Read the model definition and answer for the solid it produces. Units are mm, in the model's axes. Face numbers are marked on the shaded views. A direction names the side the tool comes from. Give positions to 0.01 mm unless a question says otherwise; leave off trailing zeros. Write each loop counter-clockwise with the first axis right and the second up, starting at its lowest first coordinate (ties: lowest second). Pieces come first, ordered by that corner, then holes. Notation, with made-up numbers: M 13,-20.75 L 44,-20.75 A17 cw 44,8.25 Z; hole C 44.5,-23.5 d11. An arc over 180 degrees is marked long. Answer as CSV lines item,"result". Start each with the question number.
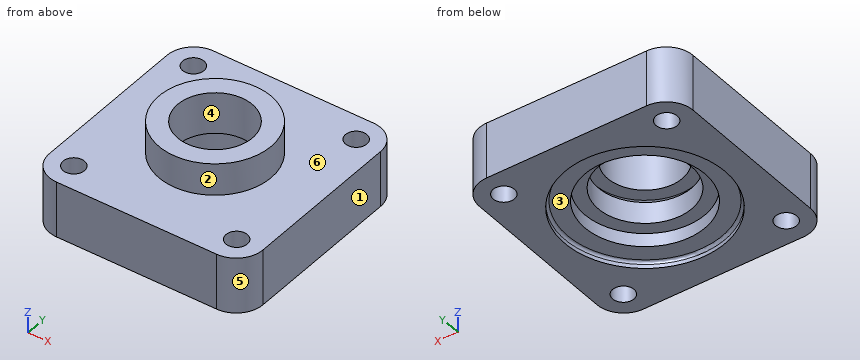
```python
from build123d import *

# Parameters (mm, degrees)
SKETCH_1_W               = 80
SKETCH_1_H               = 80
EXTRUDE_1_DEPTH          = 21
SKETCH_2_R               = 21
EXTRUDE_2_DEPTH          = 12
FILLET_1_R               = 10
SKETCH_6_R               = 4
CUT_EXTRUDE_1_DEPTH      = 21
MIRROR_2_COPY_1_SKETCH_R = 4
MIRROR_2_COPY_1_DEPTH    = 21
FILLET_2_R               = 1
FILLET_3_R               = 1


with BuildPart() as part:
    # 草图1 → 凸台-拉伸1 (new body)
    with BuildSketch(Plane.XY):
        Rectangle(SKETCH_1_W, SKETCH_1_H)
    extrude(amount=EXTRUDE_1_DEPTH)

    # 草图2 → 凸台-拉伸2 (add)
    with BuildSketch(Plane.XY.offset(21)):
        Circle(SKETCH_2_R)
    extrude(amount=EXTRUDE_2_DEPTH)

    # 草图3 → 切除-旋转1 (revolve, cut)
    with BuildSketch(Plane(origin=(0, 0, 0), x_dir=(1, 0, 0), z_dir=(0, 1, 0)), mode=Mode.PRIVATE) as cut_revolve_1_sk:
        Polygon((30, 0), (30, -2.5), (22.5, -2.5), (22.5, -7.5), (17.5, -7.5), (17.5, -15.5), (20, -15.5), (20, -17.5), (14, -17.5), (14, -33), (0, -33), (0, 0), align=None)
    revolve(cut_revolve_1_sk.sketch.rotate(Axis((0, 0, 0), (0, 0, 1)), 180), axis=Axis((0, 0, 0), (0, 0, 1)), mode=Mode.SUBTRACT)

    # 圆角1
    fillet_1_edges = [part.edges().sort_by_distance(p)[0] for p in [
        (40, -40, 10.5),
        (-40, -40, 10.5),
        (-40, 40, 10.5),
        (40, 40, 10.5),
    ]]
    fillet(fillet_1_edges, radius=FILLET_1_R)

    # 草图6 → 切除-拉伸1 (cut)
    with BuildSketch(Plane.XY.offset(21)):
        with Locations((-30.5, 30.5)):
            Circle(SKETCH_6_R)
    cut_extrude_1 = extrude(amount=-CUT_EXTRUDE_1_DEPTH, mode=Mode.SUBTRACT)

    # 镜向1: 切除-拉伸1 across plane
    add(cut_extrude_1.mirror(Plane.ZX), mode=Mode.SUBTRACT)

    # 镜向2: 切除-拉伸1 across plane
    add(cut_extrude_1.mirror(Plane(origin=(0, 0, 0), x_dir=(0, 0, 1), z_dir=(1, 0, 0))), mode=Mode.SUBTRACT)

    # 镜向2 copy 1 sketch → 镜向2 copy 1 (cut)
    with BuildSketch(Plane(origin=(0, 0, 21), x_dir=(-1, 0, 0), z_dir=(0, 0, 1))):
        with Locations((-30.5, 30.5)):
            Circle(MIRROR_2_COPY_1_SKETCH_R)
    extrude(amount=-MIRROR_2_COPY_1_DEPTH, mode=Mode.SUBTRACT)

    # 圆角2
    fillet_2_edges = [part.edges().sort_by_distance(p)[0] for p in [
        (30, 0, 2.5),
    ]]
    fillet(fillet_2_edges, radius=FILLET_2_R)

    # 圆角3
    fillet_3_edges = [part.edges().sort_by_distance(p)[0] for p in [
        (20, 0, 17.5),
    ]]
    fillet(fillet_3_edges, radius=FILLET_3_R)


solid = part.part
```
1. Find the intervals of material crossed by line 1 (Y direction, x = -30.5, z = 12.25); line 2 (X direction, y = 30, z = 12); line 3 (X direction, y = -32, z = 18.5), in increasing order. Write a range as [from, to].
2. Determine the mould class of the marked faces 4, 5 and 6 for opening direction Y: +Y half, -Y half, draft (parallel to the pull), parting line (faces both ways), or undercut.
3. Given pin 1 (19 mm diameter, centred on x = 3.5, y = -9, fed in from -Z); pin 2 (4 mm diameter, centred on x = -31.5, y = -7.5, fed in from +Z); pin 3 (6.5 mm diameter, centred on x = 30.5, y = 30.5, fed in from +Z); pin 4 (5 mm diameter, centred on y = -15, z = 26, fed in from +X), each flat-ended and moving along its own axis, determine where each tip first touches the part or whether it passes through.
4. Find section D-D on x = 31.5. Determine the outline of the cut face in (y, z).
5. For the marked faces 1, 2 and 3, determine the directions among +Z, -Z, +X, -X, +Y, -Y from which every point of the face is accessible in a straight line to the end or side of a thin tool.
6. Find section A-A on z = 6.5. Determine the outline of the cut face in (x, y), then the cut area to 3 significant figures.
Computed:
1,line 1,"y = [-39.99, -34.5], [-26.5, 26.5], [34.5, 39.99]"
1,line 2,"x = [-40, -34.47], [-26.53, 26.53], [34.47, 40]"
1,line 3,"x = [-39.8, -34.21], [-26.79, 26.79], [34.21, 39.8]"
2,face 4,"undercut"
2,face 5,"-Y half"
2,face 6,"draft"
3,pin 1,"stops at z = 7.5"
3,pin 2,"stops at z = 21"
3,pin 3,"passes through"
3,pin 4,"stops at x = 16.87"
4,outline,"M -39.89,0 L -34.37,0 L -34.37,21 L -39.89,21 Z; M -26.63,0 L 26.63,0 L 26.63,21 L -26.63,21 Z; M 34.37,0 L 39.89,0 L 39.89,21 L 34.37,21 Z"
5,face 1,"+Z, -Z, +X, +Y, -Y"
5,face 2,"+Z"
5,face 3,"-Z"
6,outline,"M -40,-30 A10 ccw -30,-40 L 30,-40 A10 ccw 40,-30 L 40,30 A10 ccw 30,40 L -30,40 A10 ccw -40,30 Z; hole C -30.5,-30.5 d8; hole C -30.5,30.5 d8; hole C 0,0 d45; hole C 30.5,-30.5 d8; hole C 30.5,30.5 d8"
6,area,"4,520 mm^2"
